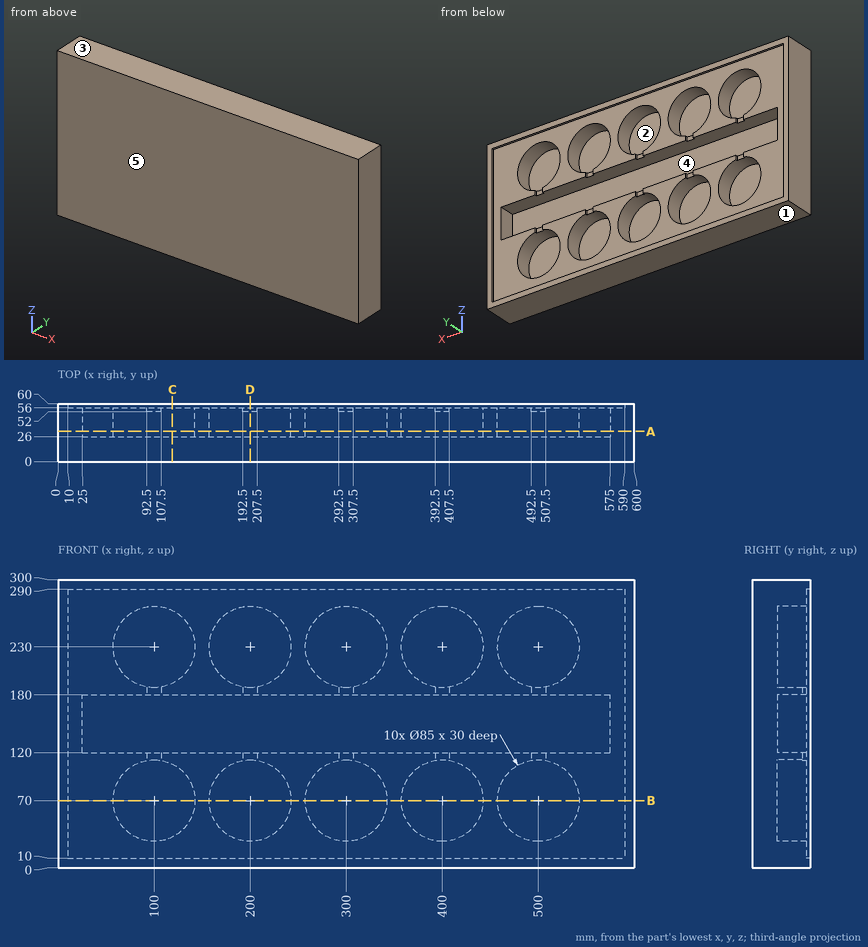
Study the drawing (mm; zero at the part's minimum x, y, z) and answer. A direction names the side the tool comes from. Round coordinates to 2 decimals unless told otherwise and drop trailing zeros. Write each loop counter-clockwise with the first axis right and the second up, starting at its lowest first coordinate (ties: lowest second). Pieces come first, ordered by that corner, then holes.
1) A cutting plane is placed at A-A on y = 31.5. Give the number of separate pieces and of enclosed holes in the cut face, and give its area (3 significant figures).
2) A cutting plane is placed at D-D on x = 200. Determine the outline of the cut face in (y, z), and give its area (3 significant figures).
3) A cutting plane is placed at B-B on z = 70. Determine the outline of the cut face in (x, y).
4) Which of the six approach directions +Z, -Z, +X, -X, +Y, -Y give full straight-line access (tool end or side, diameter ignored) to the marked faces 1 and 2?
5) A cutting plane is placed at C-C on x = 119. Determine the outline of the cut face in (y, z), and give its area (3 significant figures).
6) Determine the mould class of the marked faces 3, 4 and 5 for opening direction Z: pulls with the +Z half, pulls with the -Z half, needs draft (parallel to the pull), parting line crosses it, or undercut.
7) Consider probe 1 along X at (y, z) = (39, 70); probe 2 along Z at (x, y) = (500, 33); probe 3 along Z at (x, y) = (31, 55.5). Determine where each line is inside the solid, lowest interval first.
8) Flat-ended cylindrical pins translate along their axes: P1, Ø8, axis at x = 296.5, z = 242.5, coming from the +Y side; P2, Ø2.5, axis at x = 500.5, z = 115, coming from the +Y side; P3, Ø10, axis at x = 155.5, z = 123.5, coming from the +Y side. Find the tip coordinate at first contact, or state that the pin passes through.
Entries:
1. separate pieces: 1
1. enclosed holes: 11
1. area: 90,300 mm2
2. outline: (0, 0) - (60, 0) - (60, 10) - (56, 10) - (56, 27.5) - (26, 27.5) - (26, 112.5) - (52, 112.5) - (52, 120) - (26, 120) - (26, 180) - (52, 180) - (52, 187.5) - (26, 187.5) - (26, 272.5) - (56, 272.5) - (56, 290) - (60, 290) - (60, 300) - (0, 300) - close
2. area: 9,920 mm2
3. outline: (0, 0) - (600, 0) - (600, 60) - (590, 60) - (590, 56) - (542.5, 56) - (542.5, 26) - (457.5, 26) - (457.5, 56) - (442.5, 56) - (442.5, 26) - (357.5, 26) - (357.5, 56) - (342.5, 56) - (342.5, 26) - (257.5, 26) - (257.5, 56) - (242.5, 56) - (242.5, 26) - (157.5, 26) - (157.5, 56) - (142.5, 56) - (142.5, 26) - (57.5, 26) - (57.5, 56) - (10, 56) - (10, 60) - (0, 60) - close
4. face 1: -Z, +X, -X, +Y, -Y
4. face 2: +Y
5. outline: (0, 0) - (60, 0) - (60, 10) - (56, 10) - (56, 31.98) - (26, 31.98) - (26, 108.02) - (56, 108.02) - (56, 120) - (26, 120) - (26, 180) - (56, 180) - (56, 191.98) - (26, 191.98) - (26, 268.02) - (56, 268.02) - (56, 290) - (60, 290) - (60, 300) - (0, 300) - close
5. area: 10,500 mm2
6. face 3: pulls with the +Z half
6. face 4: undercut
6. face 5: needs draft
7. probe 1: x = 0 to 57.5, 142.5 to 157.5, 242.5 to 257.5, 342.5 to 357.5, 442.5 to 457.5, 542.5 to 600
7. probe 2: z = 0 to 27.5, 112.5 to 120, 180 to 187.5, 272.5 to 300
7. probe 3: z = 0 to 120, 180 to 300
8. P1: stops at y = 26
8. P2: stops at y = 52
8. P3: stops at y = 56
